```python
from build123d import *

# Parameters (mm, degrees)
SKETCH1_R           = 3
BOSS_EXTRUDE1_DEPTH = 2


with BuildPart() as part:
    # Sketch1 → Boss-Extrude1 (new body)
    with BuildSketch(Plane.XY):
        with BuildLine():
            Line((0, 9), (55.234065112, 6.728534899))
            Line((55.234065112, 6.728534899), (115.234079808, 6.728534899))
            ThreePointArc((115.234079808, 6.728534899), (124.234079808, -2.271465101), (115.234079808, -11.271465101))
            Line((115.234079808, -11.271465101), (55.234065112, -11.271465101))
            Line((55.234065112, -11.271465101), (0, -9))
            ThreePointArc((0, -9), (-9, 0), (0, 9))
        make_face()
        Circle(SKETCH1_R, mode=Mode.SUBTRACT)
        with Locations((55.234065112, -2.271465101)):
            Circle(SKETCH1_R, mode=Mode.SUBTRACT)
        with Locations((115.234079808, -2.271465101)):
            Circle(SKETCH1_R, mode=Mode.SUBTRACT)
        with Locations((27.617032556, -1.13573255)):
            Circle(SKETCH1_R, mode=Mode.SUBTRACT)
        with Locations((85.23407246, -2.271465101)):
            Circle(SKETCH1_R, mode=Mode.SUBTRACT)
    extrude(amount=BOSS_EXTRUDE1_DEPTH)


solid = part.part
```
Source: CAD feature listing. Evaluate the final solid. Frame: model axes, mm. Round coordinates to 2 decimals unless told otherwise and drop trailing zeros. Loops run counter-clockwise (first coordinate to the right, second up) from the corner with the lowest first, then second, coordinate; pieces in that order, holes last. Notation, with made-up numbers: M 49,19 L 103,19 A29 cw 103,48 Z; hole C 22,4 d9. An arc over 180 degrees is marked long. Use a Markdown table: item, result. Add a question column.
1. Cut plane A-A, the plane z = 1.3. Output: boundary loops of the cut face in (x, y).
2. Cut plane B-B, the plane x = 80. Output: boundary loops of the cut face in (y, z), and give its area (3 significant figures).
3. Ray query, line 1 along X through (y, z) = (-4.25, 0.6); line 2 along X through (y, z) = (-0.5, 1.75); line 3 along X through (y, z) = (-0.25, 1.55). Return the intervals inside material, ascending. Write a range as [from, to].
4. Cut plane C-C, the plane y = -7. Output: boundary loops of the cut face in (x, z).
5. Pull-direction query (Y, two-part tool) for faces 1 (the cylindrical face through (124.23, -2.07, 0.99)), 2 (the flat face through (28, -10.15, 0.99)), 3 (the cylindrical face through (30.39, -2.28, 0.99)), 4 (the flat face through (27.23, 7.88, 0.99)); classes: +Y half, -Y half, draft (parallel to the pull), parting line (faces both ways), or undercut.
6. Contact query for flat-ended pins moving along their axis: pin 1 (0.6 mm diameter, centred on x = 96.5, z = 1, fed in from +Y); pin 2 (1.5 mm diameter, centred on x = 84, y = 2.5, fed in from -Z). Output: stop coordinate, or through.
Solution:
| question | item | result |
|---|---|---|
| 1 | outline | M 0,-9 L 55.23,-11.27 L 115.23,-11.27 A9 ccw 115.23,6.73 L 55.23,6.73 L 0,9 A9 ccw Z; hole C 0,0 d6; hole C 27.62,-1.14 d6; hole C 55.23,-2.27 d6; hole C 85.23,-2.27 d6; hole C 115.23,-2.27 d6 |
| 2 | outline | M -11.27,0 L 6.73,0 L 6.73,2 L -11.27,2 Z |
| 2 | area | 36.0 mm2 |
| 3 | line 1 | x = [-7.93, 52.98], [57.49, 82.98], [87.49, 112.98], [117.49, 124.01] |
| 3 | line 2 | x = [-8.99, -2.96], [2.96, 24.69], [30.55, 52.81], [57.66, 82.81], [87.66, 112.81], [117.66, 124.06] |
| 3 | line 3 | x = [-9, -2.99], [2.99, 24.75], [30.48, 53.02], [57.45, 83.02], [87.45, 113.02], [117.45, 124] |
| 4 | outline | M -5.66,0 L 122.89,0 L 122.89,2 L -5.66,2 Z |
| 5 | face 1 | parting line |
| 5 | face 2 | -Y half |
| 5 | face 3 | undercut |
| 5 | face 4 | +Y half |
| 6 | pin 1 | stops at y = 6.73 |
| 6 | pin 2 | stops at z = 0 |
